The listing builds one solid part. Answer for the finished solid, in the listing's coordinates (mm). A direction names the side the tool comes from. Round coordinates to 2 decimals unless told otherwise and drop trailing zeros. Order: outer loops, then holes, each group sorted by start corner. A loop starts at its lowest first (then second) coordinate and runs counter-clockwise, first axis right, second up. Notation, with made-up numbers: M 8,47.5 L 42,47.5 A11 cw 42,61.5 Z; hole C 38,77 d10. An arc over 180 degrees is marked long. Put each result on its own line as item: value. Start each with the question number.
1. The part is cut by section B-B (y = 44.5). Give the vertices of the cut face in (x, z), then the cut area to 3 significant figures.
2. Each of these flat-tipped pins is pushed along its axis until it touches: pin 1 Ø8 at (x, y) = (40.5, 9) entering from +Z; pin 2 Ø1.5 at (x, y) = (103, 6) entering from +Z; pin 3 Ø12 at (y, z) = (40, 23) entering from +X; pin 4 Ø3 at (y, z) = (39, 33.5) entering from +X. Where does it stop, or does it pass through?
3. The part is cut by section A-A (z = 43.5). Give the vertices of the cut face in (x, y), then the cut area to 3 significant figures.
4. The mould has two halves that part along X. Classify faces 4 (the face through (-46.463, 35.994, 37.185)), 5 (the face through (150, 50, 0)), 6 (the face through (-18.149, 12.473, 5.972)): +X half, -X half, draft (parallel to the pull), parting line (faces both ways), or undercut.
5. Consider line 1 (Z direction, x = 126, y = 1); line 2 (X direction, y = 2, z = 1); line 3 (X direction, y = 24.5, z = 41). Determine where each line is inside the solid, lowest interval first.
6. Which of the six approach directions +Z, -Z, +X, -X, +Y, -Y give full straight-line access (tool end or side, diameter ignored) to faces 1 (the face through (70.64, -5.78, 1.61)), 2 (the face through (155.78, 32.75, 1.61)), 3 (the face through (-46, 30, 60))?
from build123d import *

# Parameters (mm, degrees)
SWEEP_1_PROFILE_R = 6


with BuildPart() as part:
    # 扫描1: sweep along a curve in space
    with BuildLine() as sweep_1_path:
        Line((150, 15, 0), (150, 50, 0))
        ThreePointArc((135, 0, 0), (145.606601718, 4.393398282, 0), (150, 15, 0))
        Line((4.442940339, 0, 0), (135, 0, 0))
        ThreePointArc((4.442940339, 0, 0), (0.182941192, 0.617635547, 0), (-3.726241034, 2.41967903, 0))
        Line((-3.726241034, 2.41967903, 0), (-33.618877196, 21.830818627, 0))
        ThreePointArc((-33.618877196, 21.830818627, 0), (-42.514507463, 27.607302173, 4.393398282), (-46.199198166, 30, 15))
        Line((-46.199198166, 30, 15), (-46.199198166, 30, 60))
    # 扫描1 profile (on start of the path) → 扫描1 (sweep)
    with BuildSketch(Plane(origin=(-46.199198166, 30, 60), x_dir=(0, -1, 0), z_dir=(0, 0, -1))):
        Circle(SWEEP_1_PROFILE_R)
    sweep(path=sweep_1_path.line)


solid = part.part
Resolved:
1. outline: C 150,0 d12
1. area: 113 mm2
2. pin 1: z = 3.32
2. pin 2: z = 2.9
2. pin 3: x = -41.73
2. pin 4: through
3. outline: C -46.2,30 d12
3. area: 113 mm2
4. face 4: parting line
4. face 5: draft
4. face 6: undercut
5. line 1: -5.92 to 5.92
5. line 2: -13.94 to 151.39
5. line 3: -48.6 to -43.8
6. face 1: none
6. face 2: +Y
6. face 3: +Z, +X, -X, +Y, -Y
